Read the model definition and answer for the solid it produces. Units are mm, in the model's axes. Face numbers are marked on the shaded views. A direction names the side the tool comes from. Coordinates: 2 decimals unless noted, no trailing zeros. Write each loop counter-clockwise with the first axis right and the second up, starting at its lowest first coordinate (ties: lowest second). Pieces come first, ordered by that corner, then holes. Notation, with made-up numbers: (-36, 7.25) -> (-31, 7.25) arc R19 cw to (-31, 28.25) -> close; hole circle Ø10 at (28.25, 64). An arc over 180 degrees is marked (long way). Return JSON: item names as keys, results as strings.
from build123d import *

# Parameters (mm, degrees)
BOSS_EXTRUDE1_DEPTH = 123
BOSS_EXTRUDE2_START = -1.2
BOSS_EXTRUDE2_DEPTH = 1.2
FILLET1_R           = 10
FILLET2_R           = 10
CUT_EXTRUDE1_DEPTH  = 318.612421042


with BuildPart() as part:
    # Sketch1 → Boss-Extrude1 (new body)
    with BuildSketch(Plane.XY):
        with BuildLine():
            Line((-86.2, -151.7), (-86.2, 150.5))
            ThreePointArc((-86.2, 150.5), (0, 236.7), (86.2, 150.5))
            Line((86.2, 150.5), (86.2, -151.7))
            Line((86.2, -151.7), (-86.2, -151.7))
        make_face()
        with BuildLine():
            Line((75, -150.5), (-75, -150.5))
            ThreePointArc((-75, -150.5), (-82.071067812, -147.571067812), (-85, -140.5))
            Line((-85, -140.5), (-85, 150.5))
            ThreePointArc((-85, 150.5), (0, 235.5), (85, 150.5))
            Line((85, 150.5), (85, -140.5))
            ThreePointArc((85, -140.5), (82.071067812, -147.571067812), (75, -150.5))
        make_face(mode=Mode.SUBTRACT)
    extrude(amount=BOSS_EXTRUDE1_DEPTH)

    # Sketch2 → Boss-Extrude2 (add)
    with BuildSketch(Plane.XY.offset(123).offset(BOSS_EXTRUDE2_START)):
        with BuildLine():
            Line((-86.2, 150.5), (-86.2, -151.7))
            Line((-86.2, -151.7), (86.2, -151.7))
            Line((86.2, -151.7), (86.2, 150.5))
            ThreePointArc((86.2, 150.5), (0, 236.7), (-86.2, 150.5))
        make_face()
    extrude(amount=BOSS_EXTRUDE2_DEPTH)

    # Fillet1
    fillet1_edges = [part.edges().sort_by_distance(p)[0] for p in [
        (-86.2, -151.7, 61.5),
    ]]
    fillet(fillet1_edges, radius=FILLET1_R)

    # Fillet2
    fillet2_edges = [part.edges().sort_by_distance(p)[0] for p in [
        (86.2, -151.7, 61.5),
    ]]
    fillet(fillet2_edges, radius=FILLET2_R)

    # Sketch3 → Cut-Extrude1 (cut, through all)
    with BuildSketch(Plane.ZY.offset(86.2)):
        with BuildLine():
            Line((8.75, 99.3), (8.75, 101.3))
            ThreePointArc((8.75, 101.3), (11.5, 104.05), (14.25, 101.3))
            Line((14.25, 101.3), (14.25, 99.3))
            ThreePointArc((14.25, 99.3), (11.5, 96.55), (8.75, 99.3))
        make_face()
        with BuildLine():
            Line((8.75, -100.7), (8.75, -98.7))
            ThreePointArc((8.75, -98.7), (11.5, -95.95), (14.25, -98.7))
            Line((14.25, -98.7), (14.25, -100.7))
            ThreePointArc((14.25, -100.7), (11.5, -103.45), (8.75, -100.7))
        make_face()
    extrude(amount=-CUT_EXTRUDE1_DEPTH, mode=Mode.SUBTRACT)


solid = part.part
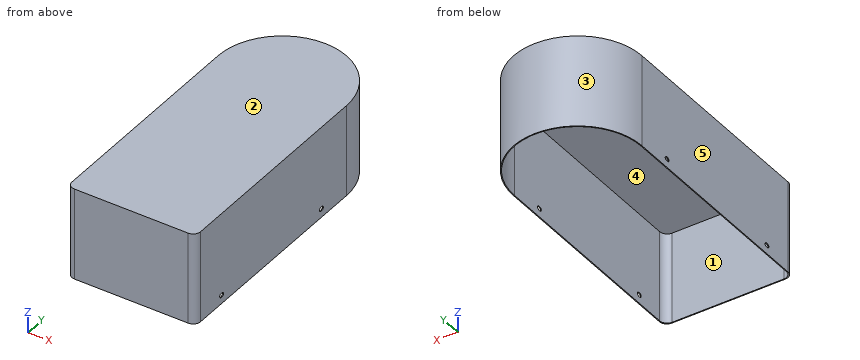
1. Flat-ended cylindrical pins translate along their axes: pin 1 Ø1.5 at (x, z) = (-50, 34) entering from +Y; pin 2 Ø4 at (x, y) = (-42, 101) entering from -Z; pin 3 Ø8 at (x, z) = (8.5, 22) entering from +Y. Find the tip coordinate at first contact, or state that the pin passes through.
Taken from the geometry:
{"pin 1": "stops at y = 221.25", "pin 2": "stops at z = 121.8", "pin 3": "stops at y = 236.58"}
2. For a pull along X with two mould halves and no side action, classify the marked faces 1, 2 and 3 as +X half, -X half, draft (parallel to the pull), parting line (faces both ways), or undercut.
Taken from the geometry:
{"face 1": "undercut", "face 2": "draft", "face 3": "parting line"}
3. A tool of negligible diameter and unlimited length cuts with its end or side. For the marked faces 4 and 5, from which of +Z, -Z, +X, -X, +Y, -Y can it reach the whole face along a straight path? Write none if from no direction.
Taken from the geometry:
{"face 4": "-Z", "face 5": "+Z, -Z, -X, +Y, -Y"}
4. The part is cut by section A-A (z = 85). Determine the outline of the cut face in (x, y).
Taken from the geometry:
{"outline": "(-86.2, -141.7) arc R10 ccw to (-76.2, -151.7) -> (76.2, -151.7) arc R10 ccw to (86.2, -141.7) -> (86.2, 150.5) arc R86.2 ccw to (-86.2, 150.5) -> close; hole (-85, -140.5) arc R10 ccw to (-75, -150.5) -> (75, -150.5) arc R10 ccw to (85, -140.5) -> (85, 150.5) arc R85 ccw to (-85, 150.5) -> close"}
5. The part is cut by section B-B (y = -66). Determine the outline of the cut face in (x, z).
Taken from the geometry:
{"outline": "(-86.2, 0) -> (-85, 0) -> (-85, 121.8) -> (85, 121.8) -> (85, 0) -> (86.2, 0) -> (86.2, 123) -> (-86.2, 123) -> close"}
6. The part is cut by section C-C (x = 7.5). Determine the outline of the cut face in (y, z), then the cut area to 3 significant figures.
Taken from the geometry:
{"outline": "(-151.7, 0) -> (-150.5, 0) -> (-150.5, 121.8) -> (235.17, 121.8) -> (235.17, 0) -> (236.37, 0) -> (236.37, 123) -> (-151.7, 123) -> close", "area": "759 mm2"}
7. Consider L1, parallel to Y at x = 2.5, z = 44; L2, parallel to X at y = -100.5, z = 71; L3, parallel to Z at x = -6, y = 104.5. Determine where each line is inside the solid, lowest interval first.
Taken from the geometry:
{"L1": "y = -151.7 to -150.5, 235.46 to 236.66", "L2": "x = -86.2 to -85, 85 to 86.2", "L3": "z = 121.8 to 123"}
